Work out the finished part from the listing and answer in its coordinate system (mm). Face numbers are marked on the shaded views. A direction names the side the tool comes from. Round coordinates to 2 decimals unless told otherwise and drop trailing zeros. Return JSON: item names as keys, results as strings.
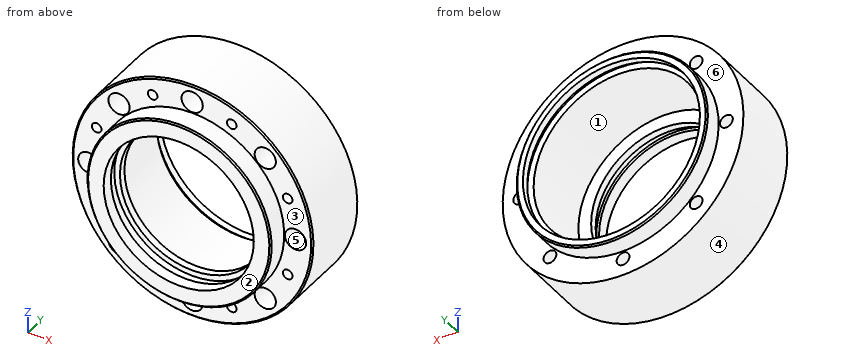
from build123d import *

# Parameters (mm, degrees)
SKETCH1_R                                          = 85
BOSS_EXTRUDE1_DEPTH                                = 50
SKETCH2_R                                          = 67.5
BOSS_EXTRUDE2_DEPTH                                = 13
SKETCH3_R                                          = 65
BOSS_EXTRUDE3_DEPTH                                = 15
CHAMFER1_SIZE                                      = 1
SKETCH4_R                                          = 52.5
CUT_EXTRUDE1_DEPTH                                 = 55
SKETCH5_R                                          = 51
CUT_EXTRUDE2_DEPTH                                 = 133.193040664
CUT_EXTRUDE3_START                                 = -8
SKETCH6_R                                          = 55
CUT_EXTRUDE3_DEPTH                                 = 8.5
HOLE_SIZE_BASED_ON_SOCKET_HEAD_CAP_SCR_D           = 9
HOLE_SIZE_BASED_ON_SOCKET_HEAD_CAP_SCR_CBORE_D     = 15
HOLE_SIZE_BASED_ON_SOCKET_HEAD_CAP_SCR_CBORE_DEPTH = 30
CIRPATTERN1_COUNT                                  = 8
CHAMFER2_SIZE                                      = 1
SKETCH15_R                                         = 55
SKETCH15_R_2                                       = 51
BOSS_EXTRUDE4_DEPTH                                = 1.5
CIRPATTERN3_COUNT                                  = 8
SKETCH20_R                                         = 53
CUT_EXTRUDE8_DEPTH                                 = 8
SKETCH22_R                                         = 60
CUT_EXTRUDE11_DEPTH                                = 58
CUT_EXTRUDE12_START                                = -8
SKETCH23_R                                         = 64.5
CUT_EXTRUDE12_DEPTH                                = 3.2
SKETCH25_R                                         = 62.5
CUT_EXTRUDE13_DEPTH                                = 8


with BuildPart() as part:
    # Sketch1 → Boss-Extrude1 (new body)
    with BuildSketch(Plane(origin=(0, 0, 0), x_dir=(1, 0, 0), z_dir=(0, 1, 0))):
        with Locations(Location((0, 0, 0), (0, 0, 270))):
            Circle(SKETCH1_R)
    extrude(amount=BOSS_EXTRUDE1_DEPTH)

    # Sketch2 → Boss-Extrude2 (add)
    with BuildSketch(Plane(origin=(0, 50, 0), x_dir=(1, 0, 0), z_dir=(0, 1, 0))):
        with Locations(Location((0, 0, 0), (0, 0, 270))):
            Circle(SKETCH2_R)
    extrude(amount=BOSS_EXTRUDE2_DEPTH)

    # Sketch3 → Boss-Extrude3 (add)
    with BuildSketch(Plane.XZ):
        with Locations(Location((0, 0, 0), (0, 0, 90))):
            Circle(SKETCH3_R)
    extrude(amount=BOSS_EXTRUDE3_DEPTH)

    # Chamfer1
    chamfer1_edges = [part.edges().sort_by_distance(p)[0] for p in [
        (0, -15, -65),
        (0, 63, -67.5),
    ]]
    chamfer(chamfer1_edges, length=CHAMFER1_SIZE)

    # Sketch4 → Cut-Extrude1 (cut)
    with BuildSketch(Plane(origin=(0, 63, 0), x_dir=(1, 0, 0), z_dir=(0, 1, 0))):
        with Locations(Location((0, 0, 0), (0, 0, 270))):
            Circle(SKETCH4_R)
    extrude(amount=-CUT_EXTRUDE1_DEPTH, mode=Mode.SUBTRACT)

    # Sketch5 → Cut-Extrude2 (cut, through all)
    with BuildSketch(Plane(origin=(0, 8, 0), x_dir=(1, 0, 0), z_dir=(0, 1, 0))):
        with Locations(Location((0, 0, 0), (0, 0, 270))):
            Circle(SKETCH5_R)
    extrude(amount=-CUT_EXTRUDE2_DEPTH, mode=Mode.SUBTRACT)

    # Sketch6 → Cut-Extrude3 (cut)
    with BuildSketch(Plane.XZ.offset(15).offset(CUT_EXTRUDE3_START)):
        with Locations(Location((0, 0, 0), (0, 0, 270))):
            Circle(SKETCH6_R)
    extrude(amount=-CUT_EXTRUDE3_DEPTH, mode=Mode.SUBTRACT)

    # Hole size (% based on socket head cap screw type)1 (through all)
    with Locations(Plane(origin=(0, 0, 0), x_dir=(-1, 0, 0), z_dir=(0, -1, 0))):
        with Locations((0, 73)):
            hole_size_based_on_socket_head_cap_scr = CounterBoreHole(HOLE_SIZE_BASED_ON_SOCKET_HEAD_CAP_SCR_D / 2, HOLE_SIZE_BASED_ON_SOCKET_HEAD_CAP_SCR_CBORE_D / 2, HOLE_SIZE_BASED_ON_SOCKET_HEAD_CAP_SCR_CBORE_DEPTH)

    # CirPattern1: Hole size (% based on socket head cap screw type)1 ×8 about axis
    cirpattern1_axis = Axis((0, 0, 0), (0, 1, 0))
    for i in range(1, CIRPATTERN1_COUNT):
        add(hole_size_based_on_socket_head_cap_scr.rotate(cirpattern1_axis, i * 360 / CIRPATTERN1_COUNT), mode=Mode.SUBTRACT)

    # Chamfer2
    chamfer2_edges = [part.edges().sort_by_distance(p)[0] for p in [
        (0, 0, -85),
    ]]
    chamfer(chamfer2_edges, length=CHAMFER2_SIZE)

    # Sketch15 → Boss-Extrude4 (add)
    with BuildSketch(Plane.XZ.offset(-1.5)):
        with Locations(Location((0, 0, 0), (0, 0, 270))):
            Circle(SKETCH15_R)
        with Locations(Location((0, 0, 0), (0, 0, 90))):
            Circle(SKETCH15_R_2, mode=Mode.SUBTRACT)
    extrude(amount=BOSS_EXTRUDE4_DEPTH)

    # Sketch19 → M8 Tapped Hole1 (revolve, cut)
    with BuildSketch(Plane(origin=(-27.935890563, 0, 67.443205873), x_dir=(0, 0, -1), z_dir=(1, 0, 0))):
        Polygon((0, 0), (0, 25.792926105), (3.4, 23.75), (3.4, 0), align=None)
    m8_tapped_hole1 = revolve(axis=Axis((-27.935890563, -6.35, 67.443205873), (0, 1, 0)), mode=Mode.SUBTRACT)

    # CirPattern3: M8 Tapped Hole1 ×8 about axis
    cirpattern3_axis = Axis((0, 0, 0), (0, 1, 0))
    for i in range(1, CIRPATTERN3_COUNT):
        add(m8_tapped_hole1.rotate(cirpattern3_axis, i * 360 / CIRPATTERN3_COUNT), mode=Mode.SUBTRACT)

    # Sketch20 → Cut-Extrude8 (cut)
    with BuildSketch(Plane.XZ.offset(15)):
        with Locations(Location((0, 0, 0), (0, 0, 270))):
            Circle(SKETCH20_R)
    extrude(amount=-CUT_EXTRUDE8_DEPTH, mode=Mode.SUBTRACT)

    # Sketch22 → Cut-Extrude11 (cut)
    with BuildSketch(Plane(origin=(0, 63, 0), x_dir=(1, 0, 0), z_dir=(0, 1, 0))):
        with Locations(Location((0, 0, 0), (0, 0, 270))):
            Circle(SKETCH22_R)
    extrude(amount=-CUT_EXTRUDE11_DEPTH, mode=Mode.SUBTRACT)

    # Sketch23 → Cut-Extrude12 (cut)
    with BuildSketch(Plane(origin=(0, 63, 0), x_dir=(1, 0, 0), z_dir=(0, 1, 0)).offset(CUT_EXTRUDE12_START)):
        with Locations(Location((0, 0, 0), (0, 0, 270))):
            Circle(SKETCH23_R)
    extrude(amount=CUT_EXTRUDE12_DEPTH, mode=Mode.SUBTRACT)

    # Sketch25 → Cut-Extrude13 (cut)
    with BuildSketch(Plane(origin=(0, 63, 0), x_dir=(1, 0, 0), z_dir=(0, 1, 0))):
        with Locations(Location((0, 0, 0), (0, 0, 270))):
            Circle(SKETCH25_R)
    extrude(amount=-CUT_EXTRUDE13_DEPTH, mode=Mode.SUBTRACT)


solid = part.part
Item 1: Each of these flat-tipped pins is pushed along its axis until it touches: pin 1 (1.5 mm diameter, centred on x = 26.5, y = 28, fed in from +Z); pin 2 (17 mm diameter, centred on x = -51.62, z = 51.62, fed in from -Y); pin 3 (6 mm diameter, centred on x = -39.5, y = 4, fed in from -Z); pin 4 (16.5 mm diameter, centred on x = 51.5, z = 49, fed in from -Y). Where does it stop, or does it pass through?
Output:
{"pin 1": "stops at z = 81.01", "pin 2": "stops at y = -14.5", "pin 3": "stops at z = -76.76", "pin 4": "stops at y = -15"}
Item 2: Consider line 1 along X through (y, z) = (46.5, -2.5); line 2 along X through (y, z) = (14, -26); line 3 along Z through (x, y) = (36, 25.5). Determine where each line is inside the solid, lowest interval first. Write a range as [from, to].
Output:
{"line 1": "x = [-84.96, -76.74], [-69.26, -59.95], [59.95, 69.26], [76.74, 84.96]", "line 2": "x = [-80.93, -70.24], [-64.65, -54.07], [54.07, 64.65], [70.24, 80.93]", "line 3": "z = [-77, -48], [48, 77]"}
Item 3: The mould has two halves that part along X. Classify the marked faces 4, 5 and 6: pulls with the +X half, pulls with the -X half, needs draft (parallel to the pull), parting line crosses it, or undercut.
Output:
{"face 4": "parting line crosses it", "face 5": "undercut", "face 6": "needs draft"}
Item 4: Which of the six approach directions +Z, -Z, +X, -X, +Y, -Y give full straight-line access (tool end or side, diameter ignored) to the marked faces 1, 2 and 3?
Output:
{"face 1": "+Y", "face 2": "+Z, -Z, +X, -X, -Y", "face 3": "-Y"}
Item 5: Find section A-A (x = 0). State how many separate pieces and enclosed holes the cut face has, plus the area to 3 significant figures.
Output:
{"separate pieces": "4", "enclosed holes": "0", "area": "1,800 mm^2"}
